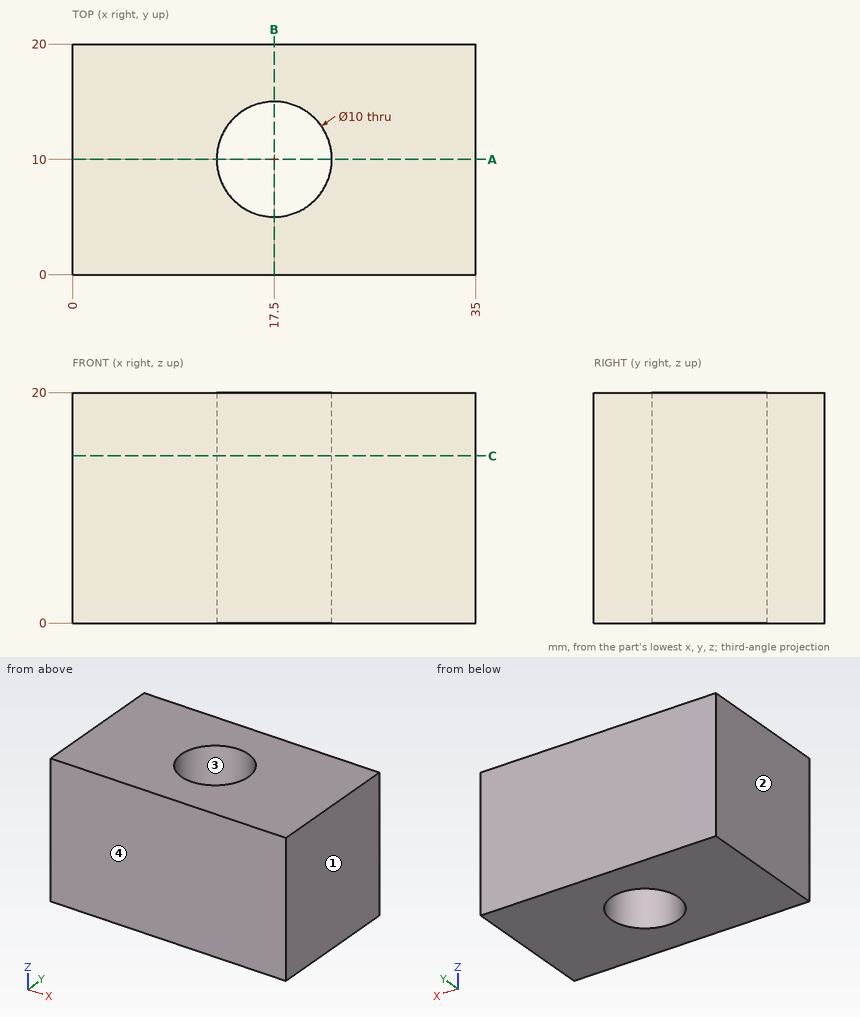
Study the drawing (mm; zero at the part's minimum x, y, z) and answer. Give positions to 0.01 mm unless a question says otherwise; leave off trailing zeros. Write each loop counter-clockwise with the first axis right and the second up, starting at its lowest first coordinate (ties: lowest second). Pieces come first, ordered by that corner, then holes. Notation, with made-up numbers: (78, -34.75) -> (97, -34.75) arc R21 cw to (97, -29.75) -> close; hole circle Ø10 at (88.5, 60.5). An arc over 180 degrees is marked (long way). Write item = value, one per line.
Q1. Consider line 1 along Y through (x, z) = (17.5, 5.5); line 2 along X through (y, z) = (13.25, 1.75); line 3 along Y through (x, z) = (19, 10). Determine where each line is inside the solid, lowest interval first.
Computed values:
line_1 = 0 to 5, 15 to 20
line_2 = 0 to 13.7, 21.3 to 35
line_3 = 0 to 5.23, 14.77 to 20
Q2. Section A-A on y = 10 is taken. Determine the outline of the cut face in (x, z), and give its area (3 significant figures).
Computed values:
outline = (0, 0) -> (12.5, 0) -> (12.5, 20) -> (0, 20) -> close; (22.5, 0) -> (35, 0) -> (35, 20) -> (22.5, 20) -> close
area = 500 mm^2
Q3. Section B-B on x = 17.5 is taken. Determine the outline of the cut face in (y, z).
Computed values:
outline = (0, 0) -> (5, 0) -> (5, 20) -> (0, 20) -> close; (15, 0) -> (20, 0) -> (20, 20) -> (15, 20) -> close
Q4. Section C-C on z = 14.5 is taken. Determine the outline of the cut face in (x, y), and give its area (3 significant figures).
Computed values:
outline = (0, 0) -> (35, 0) -> (35, 20) -> (0, 20) -> close; hole circle Ø10 at (17.5, 10)
area = 621 mm^2
Q5. For a pull along X with two mould halves and no side action, classify the marked faces 1, 2, 3 and 4 as pulls with the +X half, pulls with the -X half, needs draft (parallel to the pull), parting line crosses it, or undercut.
Computed values:
face_1 = pulls with the +X half
face_2 = pulls with the -X half
face_3 = undercut
face_4 = needs draft
